from build123d import *

# Parameters (mm, degrees)
SKETCH_1_W                   = 50
SKETCH_1_H                   = 45
EXTRUDE_1_DEPTH              = 10
SKETCH_6_W                   = 50
SKETCH_6_H                   = 17
EXTRUDE_2_DEPTH              = 25
CHAMFER_1_SIZE               = 2
HOLE_WIZARD_1_AT_2_COUNT     = 2
HOLE_WIZARD_1_AT_2_PITCH     = 40
HOLE_WIZARD_2_AT_2_COUNT     = 2
HOLE_WIZARD_2_AT_2_PITCH     = 40
HOLE_WIZARD_M4_1_D           = 3.3
HOLE_WIZARD_M4_1_CSINK_D     = 4.05
HOLE_WIZARD_M4_1_CSINK_ANGLE = 90


with BuildPart() as part:
    # 草图1 → 凸台-拉伸1 (new body)
    with BuildSketch(Plane.XY):
        with Locations((-25, 22.5)):
            Rectangle(SKETCH_1_W, SKETCH_1_H)
    extrude(amount=EXTRUDE_1_DEPTH)

    # 草图6 → 凸台-拉伸2 (add)
    with BuildSketch(Plane.XY.offset(10)):
        with Locations((-25, 8.5)):
            Rectangle(SKETCH_6_W, SKETCH_6_H)
    extrude(amount=EXTRUDE_2_DEPTH)

    # 倒角1
    chamfer_1_edges = [part.edges().sort_by_distance(p)[0] for p in [
        (0, 0, 17.5),
        (-50, 0, 17.5),
        (-50, 45, 5),
        (0, 45, 5),
    ]]
    chamfer(chamfer_1_edges, length=CHAMFER_1_SIZE)

    # 草图4 → 打孔尺寸(%根据)内六角圆柱头螺钉的类型1 (revolve, cut)
    with BuildSketch(Plane(origin=(-45, 36.5, 10), x_dir=(0, -1, 0), z_dir=(1, 0, 0))):
        Polygon((0, 0), (0, 11.291850331), (2.15, 10), (2.15, 4.6), (4, 4.6), (4, 0.3), (4.3, 0), align=None)
    hole_wizard_1 = revolve(axis=Axis((-45, 36.5, 16.35), (0, 0, -1)), mode=Mode.SUBTRACT)

    # 打孔尺寸(%根据)内六角圆柱头螺钉的类型1 at 2: 打孔尺寸(%根据)内六角圆柱头螺钉的类型1 ×2
    with Locations(*[(i * HOLE_WIZARD_1_AT_2_PITCH, 0, 0) for i in range(1, HOLE_WIZARD_1_AT_2_COUNT)]):
        add(hole_wizard_1, mode=Mode.SUBTRACT)

    # 草图8 → 打孔尺寸(%根据)内六角圆柱头螺钉的类型2 (revolve, cut)
    with BuildSketch(Plane(origin=(-45, 8.5, 35), x_dir=(0, -1, 0), z_dir=(1, 0, 0))):
        Polygon((0, 0), (0, 35), (2.15, 35), (2.15, 25), (4, 25), (4, 0.3), (4.3, 0), align=None)
    hole_wizard_2 = revolve(axis=Axis((-45, 8.5, 41.35), (0, 0, -1)), mode=Mode.SUBTRACT)

    # 打孔尺寸(%根据)内六角圆柱头螺钉的类型2 at 2: 打孔尺寸(%根据)内六角圆柱头螺钉的类型2 ×2
    with Locations(*[(i * HOLE_WIZARD_2_AT_2_PITCH, 0, 0) for i in range(1, HOLE_WIZARD_2_AT_2_COUNT)]):
        add(hole_wizard_2, mode=Mode.SUBTRACT)

    # M4 螺纹孔1 (through all)
    with Locations(Plane(origin=(0, 17, 0), x_dir=(1, 0, 0), z_dir=(0, 1, 0))):
        with Locations((-35, -25), (-15, -25)):
            CounterSinkHole(HOLE_WIZARD_M4_1_D / 2, HOLE_WIZARD_M4_1_CSINK_D / 2, counter_sink_angle=HOLE_WIZARD_M4_1_CSINK_ANGLE)


solid = part.part
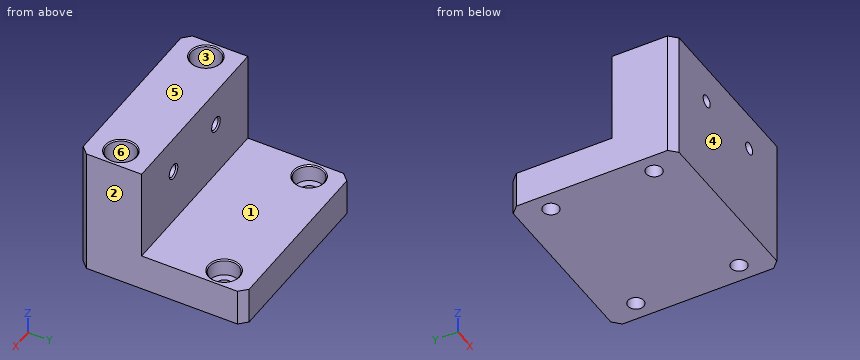
Can you work these out from the model? Positions are in its coordinate system, mm. Face numbers are marked on the shaded views. A direction names the side the tool comes from. Give positions to 0.01 mm unless a question says otherwise; leave off trailing zeros. Order: outer loops, then holes, each group sorted by start corner. A loop starts at its lowest first (then second) coordinate and runs counter-clockwise, first axis right, second up. Notation, with made-up numbers: M -5,45.25 L 36,45.25 A28 ccw 36,75.25 Z; hole C 30.5,71 d11. An arc over 180 degrees is marked long. Use a Markdown table: item, result. Add a question column.
Item 1: Will these pins go through, and if not, where does the flat tip stop? pin 1 (12 mm diameter, centred on x = -24, y = 30.5, fed in from +Z); pin 2 (4 mm diameter, centred on x = -15, z = 25, fed in from -Y); pin 3 (4 mm diameter, centred on x = -6, y = 38, fed in from +Z); pin 4 (4 mm diameter, centred on x = -35, z = 25, fed in from +Y) (3 decimals).
Item 2: Suppose I cut it at A-A (z = 25). List the corners of the cut face in (x, y) for me (3 decimals).
Item 3: We'd pull the mould along Y, two halves only. Please class the marked faces 4, 5 and 6: +Y half, -Y half, draft (parallel to the pull), parting line (faces both ways), or undercut.
Item 4: Suppose I cut it at D-D (z = 14). List the corners of the cut face in (x, y) for me, then the cut area to 3 significant figures.
Item 5: Suppose I cut it at B-B (x = -5). List the corners of the cut face in (y, z) for me, then the cut area to 3 significant figures.
Item 6: If I drill on L1, parallel to X at y = 8.5, z = 3.5; L2, parallel to Y at x = -45, z = 8; L3, parallel to Y at x = -5, z = 25.5, over which ranges is the centre line in solid material (lowest first)? Write a range as [from, to].
Item 7: For the marked faces 1, 2 and 3, which set-ups out of +Z, -Z, +X, -X, +Y, -Y let a thin tool reach every point of the face, with its end or its side?
Item 8: Suppose I cut it at C-C (y = 8.5). List the corners of the cut face in (x, z) for me.
Answer sheet:
| question | item | result |
|---|---|---|
| 1 | pin 1 | stops at z = 10 |
| 1 | pin 2 | stops at y = 0 |
| 1 | pin 3 | stops at z = 5.4 |
| 1 | pin 4 | stops at y = 16.975 |
| 2 | outline | M -50,2 L -48,0 L -36.65,0 L -36.65,16.625 L -37.025,17 L -50,17 Z; M -33.35,0 L -16.65,0 L -16.65,16.625 L -17.025,17 L -32.975,17 L -33.35,16.625 Z; M -13.35,0 L -2,0 L 0,2 L 0,17 L -12.975,17 L -13.35,16.625 Z; hole C -45,8.5 d8; hole C -5,8.5 d8 |
| 3 | face 4 | -Y half |
| 3 | face 5 | draft |
| 3 | face 6 | undercut |
| 4 | outline | M -50,2 L -48,0 L -2,0 L 0,2 L 0,17 L -50,17 Z; hole C -45,8.5 d8; hole C -5,8.5 d8 |
| 4 | area | 745 mm² |
| 5 | outline | M 0,0 L 6.35,0 L 6.35,10 L 4.5,10 L 4.5,34.7 L 4.2,35 L 0,35 Z; M 10.65,0 L 34.35,0 L 34.35,5.4 L 32.5,5.4 L 32.5,9.7 L 32.2,10 L 17,10 L 17,35 L 12.8,35 L 12.5,34.7 L 12.5,10 L 10.65,10 Z; M 38.65,0 L 45,0 L 45,10 L 40.8,10 L 40.5,9.7 L 40.5,5.4 L 38.65,5.4 Z |
| 5 | area | 572 mm² |
| 6 | L1 | x = [-50, -47.15], [-42.85, -7.15], [-2.85, 0] |
| 6 | L2 | y = [0, 6.35], [10.65, 32.5], [40.5, 45] |
| 6 | L3 | y = [0, 4.5], [12.5, 17] |
| 7 | face 1 | +Z, +X, -X, +Y |
| 7 | face 2 | +Z, -Z, +X, +Y, -Y |
| 7 | face 3 | +Z |
| 8 | outline | M -50,0 L -47.15,0 L -47.15,10 L -49,10 L -49,34.7 L -49.3,35 L -50,35 Z; M -42.85,0 L -7.15,0 L -7.15,10 L -9,10 L -9,34.7 L -9.3,35 L -40.7,35 L -41,34.7 L -41,10 L -42.85,10 Z; M -2.85,0 L 0,0 L 0,35 L -0.7,35 L -1,34.7 L -1,10 L -2.85,10 Z; hole C -35,25 d3.3; hole C -15,25 d3.3 |
